Geometry check sheet. Reference: drawing and pictorial views, mm from the part's lowest x, y, z. Give positions to 0.01 mm unless a question says otherwise; leave off trailing zeros. Write each loop counter-clockwise with the first axis right and the second up, starting at its lowest first coordinate (ties: lowest second). Pieces come first, ordered by that corner, then holes. Notation, with made-up numbers: (83.25, 17.5) - (132.25, 17.5) arc R22 cw to (132.25, 39.5) - close; hole circle Ø9 at (75, 79.25). An arc over 180 degrees is marked (long way). Write item = value, one per line. Start each with the question number.
(1) Section check B-B, the plane x = 85. Enter the section's corners in (y, z), plus the area to 3 significant figures.
(2) Section check C-C, the plane z = 10.75. Enter the section's corners in (x, y).
(3) Depth check by flat-ended pin: pin 1 Ø6 at (x, y) = (20, 40) entering from -Z. Enter the tip coordinate at first touch or a pass-through.
(4) Thickness scan on L1, parallel to Y at x = 85, z = 7.5; L2, parallel to X at y = 37.5, z = 8.25; L3, parallel to X at y = 41.5, z = 4. Record the ranges inside material, lowest first.
(5) Section check A-A, the plane y = 40. Enter the section's corners in (x, z), plus the area to 3 significant figures.
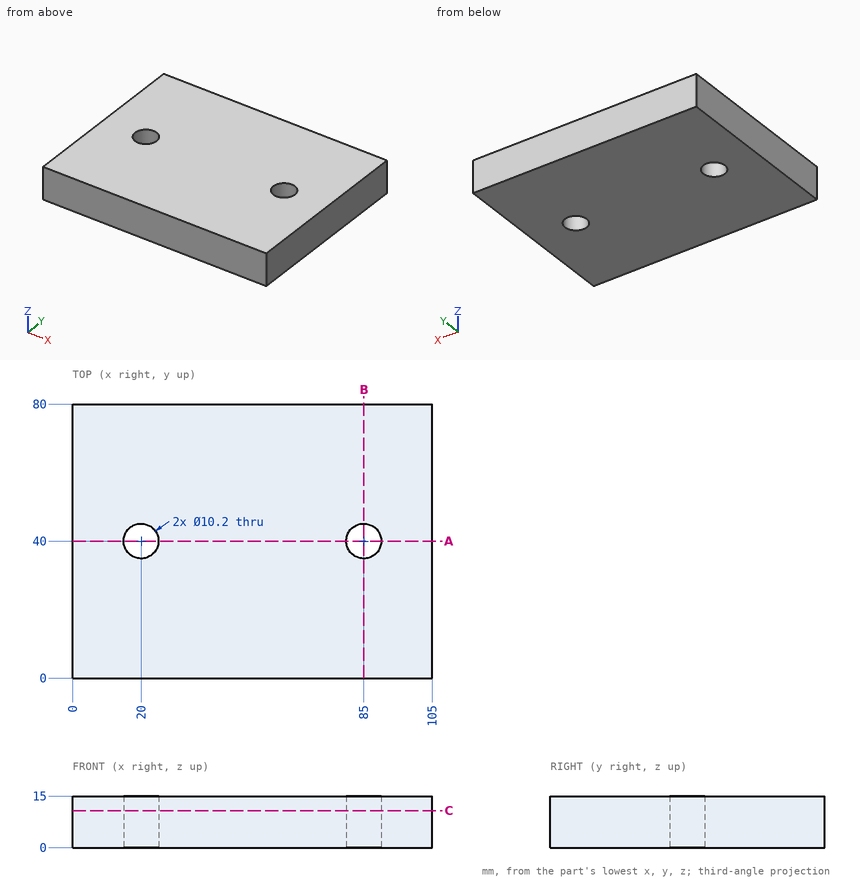
Model answer:
q1.outline = (0, 0) - (34.9, 0) - (34.9, 15) - (0, 15) - close; (45.1, 0) - (80, 0) - (80, 15) - (45.1, 15) - close
q1.area = 1,050 mm²
q2.outline = (0, 0) - (105, 0) - (105, 80) - (0, 80) - close; hole circle Ø10.2 at (20, 40); hole circle Ø10.2 at (85, 40)
q3.pin_1 = through
q4.L1 = 0 to 34.9, 45.1 to 80
q4.L2 = 0 to 15.55, 24.45 to 80.55, 89.45 to 105
q4.L3 = 0 to 15.13, 24.87 to 80.13, 89.87 to 105
q5.outline = (0, 0) - (14.9, 0) - (14.9, 15) - (0, 15) - close; (25.1, 0) - (79.9, 0) - (79.9, 15) - (25.1, 15) - close; (90.1, 0) - (105, 0) - (105, 15) - (90.1, 15) - close
q5.area = 1,270 mm²
